Could you check a few things on this drawing? It's one solid part, dimensions in mm from its lowest x, y, z. A direction names the side the tool comes from. Round coordinates to 2 decimals unless told otherwise and drop trailing zeros. Loops run counter-clockwise (first coordinate to the right, second up) from the corner with the lowest first, then second, coordinate; pieces in that order, holes last. Notation, with made-up numbers: M 36,6 L 73,6 A28 ccw 73,31 Z; hole C -26.5,-1.5 d11. An arc over 180 degrees is marked long. Return JSON: item names as keys, results as strings.
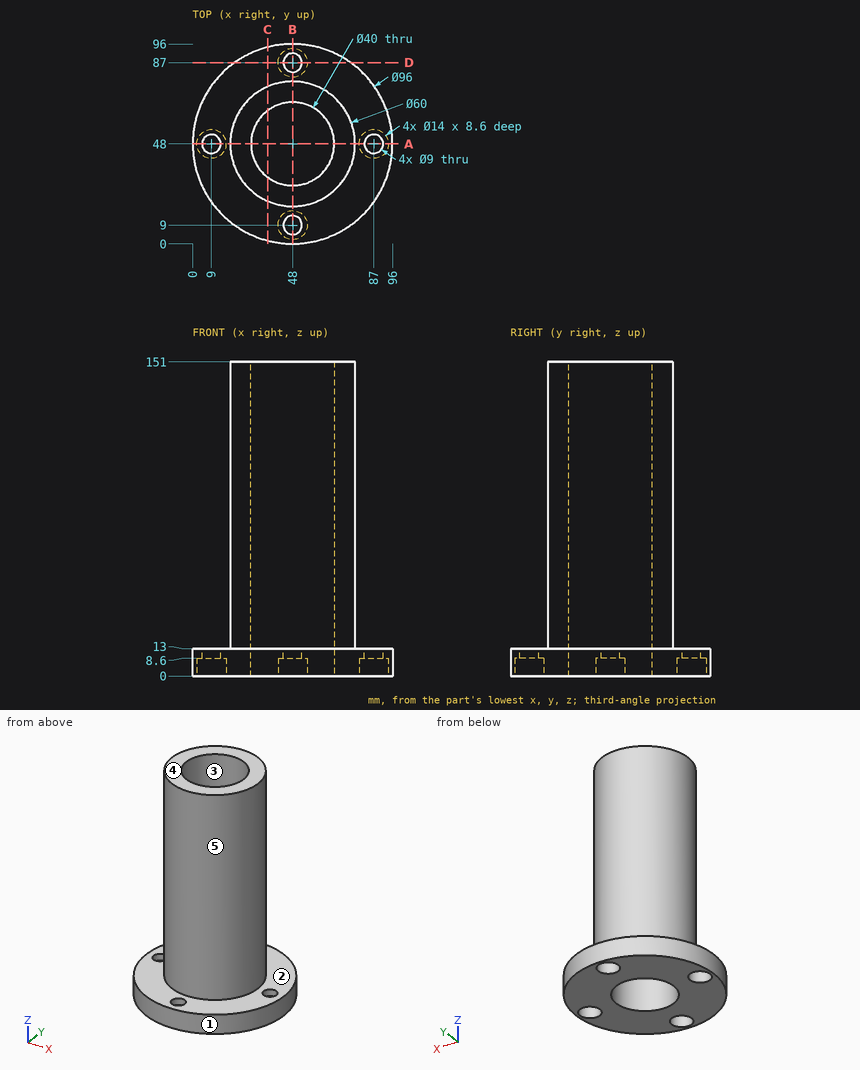
Q1. Suppose I cut it at D-D, the plane y = 87. Please give me the cut outline in (x, z).
Results:
{"outline": "M 20.02,0 L 41,0 L 41,8.6 L 43.5,8.6 L 43.5,13 L 20.02,13 Z; M 52.5,8.6 L 55,8.6 L 55,0 L 75.98,0 L 75.98,13 L 52.5,13 Z"}
Q2. On a 3-axis mill with a long thin cutter (end or side, diameter ignored), from which of +Z, -Z, +X, -X, +Y, -Y can I reach the whole of each face in a straight line? I mean the marked faces 1 and 2. Say none if no direction works.
Results:
{"face 1": "+Z, -Z", "face 2": "+Z"}
Q3. Suppose I cut it at C-C, the plane x = 36. Please give me the cut outline in (y, z).
Results:
{"outline": "M 1.52,0 L 32,0 L 32,151 L 20.5,151 L 20.5,13 L 1.52,13 Z; M 64,0 L 94.48,0 L 94.48,13 L 75.5,13 L 75.5,151 L 64,151 Z"}
Q4. Thinking about a two-plate mould opening in X: for the marked faces 3, 4 and 5, which applies, pulls with the +X half, pulls with the -X half, needs draft (parallel to the pull), parting line crosses it, or undercut?
Results:
{"face 3": "undercut", "face 4": "needs draft", "face 5": "parting line crosses it"}
Q5. Suppose I cut it at A-A, the plane y = 48. Please give me the cut outline in (x, z), plus the area to 3 significant figures.
Results:
{"outline": "M 0,0 L 2,0 L 2,8.6 L 4.5,8.6 L 4.5,13 L 0,13 Z; M 13.5,8.6 L 16,8.6 L 16,0 L 28,0 L 28,151 L 18,151 L 18,13 L 13.5,13 Z; M 68,0 L 80,0 L 80,8.6 L 82.5,8.6 L 82.5,13 L 78,13 L 78,151 L 68,151 Z; M 91.5,8.6 L 94,8.6 L 94,0 L 96,0 L 96,13 L 91.5,13 Z", "area": "3,170 mm2"}
Q6. If I drill on line 1 along Y through (x, z) = (48, 12.1); line 2 along Y through (x, z) = (48, 5.25); line 3 along Y through (x, z) = (48, 34.5), over which ranges is the centre line in solid material (lowest first)?
Results:
{"line 1": "y = 0 to 4.5, 13.5 to 28, 68 to 82.5, 91.5 to 96", "line 2": "y = 0 to 2, 16 to 28, 68 to 80, 94 to 96", "line 3": "y = 18 to 28, 68 to 78"}
Q7. I'm going to push flat-ended pins straight in: pin 1 Ø6 at (x, z) = (41, 81.5) entering from -Y; pin 2 Ø7 at (x, y) = (85.5, 48.5) entering from -Z; pin 3 Ø3 at (y, z) = (69.5, 84) entering from +X. Where does each tip first touch, or does it pass through?
Results:
{"pin 1": "stops at y = 18.27", "pin 2": "stops at z = 8.6", "pin 3": "stops at x = 70.36"}
